The model under review builds one solid part; all positions refer to its coordinate system, in mm. A direction names the side the tool comes from. Give positions to 0.01 mm unless a question says otherwise; leave off trailing zeros. Loops run counter-clockwise (first coordinate to the right, second up) from the corner with the lowest first, then second, coordinate; pieces in that order, holes last. Notation, with made-up numbers: M 78,63.5 L 113,63.5 A10 ccw 113,74.5 Z; hole C 18,51.25 d6. An arc over 180 degrees is marked long. One line per item, written item: value. Start each with the question number.
Q1. To check wall thickness, follow line 1 along Y through (x, z) = (2.1, 37.5); line 2 along Y through (x, z) = (4, -34.5); line 3 along Z through (x, y) = (6, 34). State the ranges of each line that lie inside material, in increasing order. Write a range as from..to.
Q2. Mouldability with a two-part tool opening along Y and no side actions: class faces 3 (the face through (10, 1, 1)), 4 (the face through (2.12, -29.879, -40.247)), 5 (the face through (5, 50, 1)) as released by +Y, released by -Y, zero draft, split by the parting line, or undercut.
Q3. For pin 1 (5 mm diameter, centred on y = 30, z = -37.5, fed in from -X); pin 2 (5 mm diameter, centred on y = 28, z = 38, fed in from +X), all flat-tipped, find the tip position at first contact; note any pin that passes through.
Q4. We need section B-B on y = 7.5. Write out the cut boundary in (x, z), plus the area to 3 significant figures.
Q5. For faces 1 (the face through (7.19, -29.781, -32.504)), 2 (the face through (4.93, 8.919, -36.048)), list the 3-axis set-ups (+Z, -Z, +X, -X, +Y, -Y) from which the entire face can be reached by the end or side of a thin tool; tool diameter is ignored.
Q6. We need section A-A on z = 37.5. Write out the cut boundary in (x, y), plus the area to 3 significant figures.
```python
from build123d import *

# Parameters (mm, degrees)
SKETCH_1_W                = 85
SKETCH_1_H                = 100
EXTRUDE_1_DEPTH           = 10
HOLE_WIZARD_1_D           = 5.5
HOLE_WIZARD_1_CBORE_D     = 10.001
HOLE_WIZARD_1_CBORE_DEPTH = 5.7
HOLE_WIZARD_M5_1_D        = 4.2


with BuildPart() as part:
    # 草图1 → 凸台-拉伸1 (new body)
    with BuildSketch(Plane(origin=(0, 0, 0), x_dir=(0, 0, -1), z_dir=(1, 0, 0))):
        Rectangle(SKETCH_1_W, SKETCH_1_H)
    extrude(amount=EXTRUDE_1_DEPTH)

    # 打孔尺寸(%根据)内六角圆柱头螺钉的类型1 (through all)
    with Locations(Plane(origin=(10, 0, 0), x_dir=(0, 0, -1), z_dir=(1, 0, 0))):
        with Locations((-37.5, 30), (-37.5, -30), (37.5, 30), (37.5, -30)):
            CounterBoreHole(HOLE_WIZARD_1_D / 2, HOLE_WIZARD_1_CBORE_D / 2, HOLE_WIZARD_1_CBORE_DEPTH)

    # M5 螺纹孔1 (through all)
    with Locations(Plane(origin=(10, 0, 0), x_dir=(0, 0, -1), z_dir=(1, 0, 0))):
        with Locations((34.5, 7.5), (34.5, -7.5)):
            Hole(HOLE_WIZARD_M5_1_D / 2)


solid = part.part
```
Solved:
1. line 1: -50..-32.75, -27.25..27.25, 32.75..50
1. line 2: -50..-9.6, -5.4..5.4, 9.6..50
1. line 3: -42.5..-40.5, -34.5..34.5, 40.5..42.5
2. face 3: zero draft
2. face 4: undercut
2. face 5: released by +Y
3. pin 1: through
3. pin 2: x = 4.3
4. outline: M 0,-42.5 L 10,-42.5 L 10,-36.6 L 0,-36.6 Z; M 0,-32.4 L 10,-32.4 L 10,42.5 L 0,42.5 Z
4. area: 808 mm2
5. face 1: +X
5. face 2: +X, -X
6. outline: M 0,-50 L 10,-50 L 10,-35 L 4.3,-35 L 4.3,-32.75 L 0,-32.75 Z; M 0,-27.25 L 4.3,-27.25 L 4.3,-25 L 10,-25 L 10,25 L 4.3,25 L 4.3,27.25 L 0,27.25 Z; M 0,32.75 L 4.3,32.75 L 4.3,35 L 10,35 L 10,50 L 0,50 Z
6. area: 839 mm2
